from build123d import *

# Parameters (mm, degrees)
GB_T_6728_2002_SQUARE_HOLLOW_SECTION_60_DEPTH = 930
CUT_EXTRUDE1_DEPTH                            = 933.416216075
CUT_EXTRUDE1_DEPTH_BACK                       = 933.416216075


with BuildPart() as part:
    # Sketch1 → GB/T 6728-2002 square hollow section 60×60×4(1) (new body)
    with BuildSketch(Plane(origin=(0, 0, 0), x_dir=(-1, 0, 0), z_dir=(0, 1, 0))):
        with BuildLine():
            Line((-22, -30), (22, -30))
            ThreePointArc((22, -30), (27.656854249, -27.656854249), (30, -22))
            Line((30, -22), (30, 22))
            ThreePointArc((30, 22), (27.656854249, 27.656854249), (22, 30))
            Line((22, 30), (-22, 30))
            ThreePointArc((-22, 30), (-27.656854249, 27.656854249), (-30, 22))
            Line((-30, 22), (-30, -22))
            ThreePointArc((-30, -22), (-27.656854249, -27.656854249), (-22, -30))
        make_face()
        with BuildLine():
            Line((-22, -26), (22, -26))
            ThreePointArc((22, -26), (24.828427125, -24.828427125), (26, -22))
            Line((26, -22), (26, 22))
            ThreePointArc((26, 22), (24.828427125, 24.828427125), (22, 26))
            Line((22, 26), (-22, 26))
            ThreePointArc((-22, 26), (-24.828427125, 24.828427125), (-26, 22))
            Line((-26, 22), (-26, -22))
            ThreePointArc((-26, -22), (-24.828427125, -24.828427125), (-22, -26))
        make_face(mode=Mode.SUBTRACT)
    extrude(amount=GB_T_6728_2002_SQUARE_HOLLOW_SECTION_60_DEPTH)

    # Sketch2 → Cut-Extrude1 (cut, two sides: drawn at the far end of the back side and taken through both)
    with BuildSketch(Plane.XY.offset(30).offset(-CUT_EXTRUDE1_DEPTH_BACK)):
        Polygon((-30, 930), (30, 899.206782946), (30, 930), align=None)
        Polygon((-30, 0), (-30, 30.793217054), (30, 0), align=None)
    extrude(amount=CUT_EXTRUDE1_DEPTH + CUT_EXTRUDE1_DEPTH_BACK, mode=Mode.SUBTRACT)


solid = part.part
Check sheet for the modelled part. Datum: model origin and axes. Units: mm. A direction names the side the tool comes from. Give positions to 0.01 mm unless a question says otherwise; leave off trailing zeros. Write each loop counter-clockwise with the first axis right and the second up, starting at its lowest first coordinate (ties: lowest second). Pieces come first, ordered by that corner, then holes. Notation, with made-up numbers: (4, -24) -> (45, -24) arc R36 cw to (45, 10) -> close; hole circle Ø8 at (-1.75, 44). An arc over 180 degrees is marked (long way). Write item = value, one per line.
Item 1: Release check for a two-part mould opening along Z. For faces 3 (the flat face through (-26, 472, 0)), 4 (the flat face through (0, 459, 30)), 5 (the flat face through (-0.4, 15.6, 26.2)) record: +Z half, -Z half, draft (parallel to the pull), parting line (faces both ways), or undercut.
Output:
face_3 = undercut
face_4 = +Z half
face_5 = draft
Item 2: Sectioned sample at B-B on z = -3.5. Record the boundary of the cut face in (x, y), and give its area (3 significant figures).
Output:
outline = (-30, 30.79) -> (-26, 28.74) -> (-26, 927.95) -> (-30, 930) -> close; (26, 2.05) -> (30, 0) -> (30, 899.21) -> (26, 901.26) -> close
area = 7,190 mm^2
Item 3: Tool access check on faces 1 (the flat face through (-30, 474, 0)), 2 (the flat face through (0, 459, 26)). Record the directions out of +Z, -Z, +X, -X, +Y, -Y that give a thin tool (end or side, any length) a straight path to the whole face; none if there is none.
Output:
face_1 = +Z, -Z, -X, +Y, -Y
face_2 = +Y, -Y
Item 4: Scan lines: probe 1 along Z at (x, y) = (12, 666); probe 2 along Z at (x, y) = (23, 550). Record each from-to range of solid material in increasing order. Write a range as from..to.
Output:
probe_1 = -30..-26, 26..30
probe_2 = -29.94..-25.87, 25.87..29.94
Item 5: Sectioned sample at C-C on x = 2. Record the boundary of the cut face in (y, z).
Output:
outline = (14.37, -30) -> (913.58, -30) -> (913.58, -26) -> (14.37, -26) -> close; (14.37, 26) -> (913.58, 26) -> (913.58, 30) -> (14.37, 30) -> close
Item 6: Gauge pin test, flat ends, axial feed: pin 1 (10 mm diameter, centred on x = -17, z = 7, fed in from +Y); pin 2 (3 mm diameter, centred on y = 622, z = 22.5, fed in from -X). Record the tip position at first contact, or that the pin passes through.
Output:
pin_1 = through
pin_2 = -30
Item 7: Sectioned sample at A-A on y = 84. Record the boundary of the cut face in (x, z).
Output:
outline = (-30, -22) arc R8 ccw to (-22, -30) -> (22, -30) arc R8 ccw to (30, -22) -> (30, 22) arc R8 ccw to (22, 30) -> (-22, 30) arc R8 ccw to (-30, 22) -> close; hole (-26, -22) arc R4 ccw to (-22, -26) -> (22, -26) arc R4 ccw to (26, -22) -> (26, 22) arc R4 ccw to (22, 26) -> (-22, 26) arc R4 ccw to (-26, 22) -> close
